```python
from build123d import *

# Parameters (mm, degrees)
SKETCH_1_W              = 23
SKETCH_1_H              = 31
SKETCH_1_R              = 7.5
EXTRUDE_1_DEPTH         = 5
CHAMFER_1_SIZE          = 4
HOLE_WIZARD_M4_1_REACH  = 35.44
HOLE_WIZARD_M4_1_BORE_R = 1.65
HOLE_WIZARD_M5_2_D      = 4.2
HOLE_WIZARD_M5_2_DEPTH  = 8.4
HOLE_WIZARD_M5_2_TIP    = 1.2618073


with BuildPart() as part:
    # 草图1 → 凸台-拉伸1 (new, symmetric)
    with BuildSketch(Plane.XY):
        with Locations((0, 15.5)):
            Rectangle(SKETCH_1_W, SKETCH_1_H)
        with Locations((0, 20)):
            Circle(SKETCH_1_R, mode=Mode.SUBTRACT)
    extrude(amount=EXTRUDE_1_DEPTH, both=True)

    # 倒角1
    chamfer_1_edges = [part.edges().sort_by_distance(p)[0] for p in [
        (11.5, 31, 0),
        (-11.5, 31, 0),
    ]]
    chamfer(chamfer_1_edges, length=CHAMFER_1_SIZE)

    # M4 螺纹孔1 bore (on position points) → M4 螺纹孔1 (cut, up to next)
    with BuildSketch(Plane.ZX.offset(31), mode=Mode.PRIVATE) as hole_wizard_m4_1_sk1:
        Circle(HOLE_WIZARD_M4_1_BORE_R)
    hole_wizard_m4_1_tool1 = extrude(hole_wizard_m4_1_sk1.sketch, amount=-HOLE_WIZARD_M4_1_REACH, mode=Mode.PRIVATE) & part.part
    add(hole_wizard_m4_1_tool1.solids().sort_by_distance((0, 31, 0))[0], mode=Mode.SUBTRACT)

    # M5 螺纹孔2
    with Locations(Plane(origin=(-6.5, 0, 0), x_dir=(0, 0, -1), z_dir=(0, -1, 0))):
        with Locations((0, 0), (0, 13)):
            Hole(HOLE_WIZARD_M5_2_D / 2, depth=HOLE_WIZARD_M5_2_DEPTH)
            with Locations((0, 0, -(HOLE_WIZARD_M5_2_DEPTH + HOLE_WIZARD_M5_2_TIP / 2))):  # 118° drill point
                Cone(0, HOLE_WIZARD_M5_2_D / 2, HOLE_WIZARD_M5_2_TIP, mode=Mode.SUBTRACT)


solid = part.part
```
Part model, mm, in its own coordinate system. A direction names the side the tool comes from. Coordinates: 2 decimals unless noted, no trailing zeros. Write each loop counter-clockwise with the first axis right and the second up, starting at its lowest first coordinate (ties: lowest second). Pieces come first, ordered by that corner, then holes.
Item 1: Slice it at A-A (y = 20). Write the cut outline in (x, z).
Item 2: Which spindle directions (+Z, -Z, +X, -X, +Y, -Y) get a long thin tool onto all of the face, cutting with end or side? Do faces 5 (the face through (-2, 31, 0)), 6 (the face through (-4.418, 4.259, -0.273)). Say none if no direction does.
Item 3: Mould opens along Z. For faces 1 (the face through (8.582, 4.259, -0.273)), 2 (the face through (0, 12, -5)), 3 (the face through (1.115, 29.184, -1.216)), 4 (the face through (11.5, 13, 0)) say: released by +Z, released by -Z, zero draft, split by the parting line, or undercut.
Item 4: Probe line 1 (X direction, y = 2.5, z = 0); line 2 (Z direction, x = -6.5, y = 3.25); line 3 (X direction, y = 6, z = 1). List the from-to ranges inside material, lowest first.
Item 5: Slice it at C-C (z = 3.5). Write the cut outline in (x, y), and give its area (3 significant figures).
Item 6: Slice it at B-B (x = 0.75). Write the cut outline in (y, z).
Item 7: Slice it at D-D (y = 7). Write the cut outline in (x, z), and give its area (3 significant figures).
Results found:
1. outline: (-11.5, -5) - (-7.5, -5) - (-7.5, 5) - (-11.5, 5) - close; (7.5, -5) - (11.5, -5) - (11.5, 5) - (7.5, 5) - close
2. face 5: +Z, -Z, +X, -X, +Y
2. face 6: -Y
3. face 1: undercut
3. face 2: released by -Z
3. face 3: undercut
3. face 4: zero draft
4. line 1: x = -11.5 to -8.6, -4.4 to 4.4, 8.6 to 11.5
4. line 2: z = -5 to -2.1, 2.1 to 5
4. line 3: x = -11.5 to -8.35, -4.65 to 4.65, 8.35 to 11.5
5. outline: (-11.5, 0) - (11.5, 0) - (11.5, 27) - (7.5, 31) - (-7.5, 31) - (-11.5, 27) - close; hole circle Ø15 at (0, 20)
5. area: 520 mm2
6. outline: (0, -5) - (12.54, -5) - (12.54, 5) - (0, 5) - close; (27.46, -5) - (31, -5) - (31, -1.47) - (27.46, -1.47) - close; (27.46, 1.47) - (31, 1.47) - (31, 5) - (27.46, 5) - close
7. outline: (-11.5, -5) - (11.5, -5) - (11.5, 5) - (-11.5, 5) - close; hole circle Ø4.2 at (-6.5, 0); hole circle Ø4.2 at (6.5, 0)
7. area: 202 mm2
